```python
from build123d import *

# Parameters (mm, degrees)
SKETCH1_R           = 17.5
SKETCH1_R_2         = 10
BOSS_EXTRUDE1_DEPTH = 25
CUT_EXTRUDE1_START  = -10
SKETCH2_R           = 17.5
SKETCH2_R_2         = 15
CUT_EXTRUDE1_DEPTH  = 10
CHAMFER1_SIZE       = 1


with BuildPart() as part:
    # Sketch1 → Boss-Extrude1 (new body)
    with BuildSketch(Plane.XY):
        Circle(SKETCH1_R)
        Circle(SKETCH1_R_2, mode=Mode.SUBTRACT)
    extrude(amount=BOSS_EXTRUDE1_DEPTH)

    # Sketch2 → Cut-Extrude1 (cut)
    with BuildSketch(Plane.XY.offset(25).offset(CUT_EXTRUDE1_START)):
        Circle(SKETCH2_R)
        Circle(SKETCH2_R_2, mode=Mode.SUBTRACT)
    extrude(amount=CUT_EXTRUDE1_DEPTH, mode=Mode.SUBTRACT)

    # Chamfer1
    chamfer1_edges = [part.edges().sort_by_distance(p)[0] for p in [
        (-15, 0, 25),
    ]]
    chamfer(chamfer1_edges, length=CHAMFER1_SIZE)


solid = part.part
```
Design review of the part built by this model. Coordinates are the model's own, in mm. A direction names the side the tool comes from. Coordinates: 2 decimals unless noted, no trailing zeros. Order: outer loops, then holes, each group sorted by start corner. A loop starts at its lowest first (then second) coordinate and runs counter-clockwise, first axis right, second up.
1) Mouldability with a two-part tool opening along Y and no side actions: class faces 1 (the cylindrical face through (-2.17, -9.76, 12.32)), 2 (the flat face through (-10, 3, 25)), 3 (the cylindrical face through (-13.887, -10.648, 7.395)) as +Y half, -Y half, draft (parallel to the pull), parting line (faces both ways), or undercut.
2) Take a section at A-A, the plane y = 0. Give the boundary of the cut face in (x, z).
3) Wall thickness on line 1 along Y through (x, z) = (0, 11.75); line 2 along Z through (x, y) = (12, -10); line 3 along Y through (x, z) = (-2, 18): over which ranges is each line inside the solid? List them lowest first.
4) Clearance check with flat-ended pins moving along their axes: pin 1 (3 mm diameter, centred on x = -9.5, z = 5.5, fed in from -Y); pin 2 (1.5 mm diameter, centred on y = -13, z = 7, fed in from -X); pin 3 (4 mm diameter, centred on x = 12, z = 21, fed in from -Y). State where each tip first meets the part, or that it passes through.
5) For faces 4 (the flat face through (13, 8, 15)), 5 (the flat face through (8, -8, 0)), list the 3-axis set-ups (+Z, -Z, +X, -X, +Y, -Y) from which the entire face can be reached by the end or side of a thin tool; tool diameter is ignored.
6) Take a section at C-C, the plane z = 20. Give the boundary of the cut face in (x, y).
Returned:
1. face 1: undercut
1. face 2: draft
1. face 3: parting line
2. outline: (-17.5, 0) - (-10, 0) - (-10, 25) - (-14, 25) - (-15, 24) - (-15, 15) - (-17.5, 15) - close; (10, 0) - (17.5, 0) - (17.5, 15) - (15, 15) - (15, 24) - (14, 25) - (10, 25) - close
3. line 1: y = -17.5 to -10, 10 to 17.5
3. line 2: z = 0 to 15
3. line 3: y = -14.87 to -9.8, 9.8 to 14.87
4. pin 1: stops at y = -15.56
4. pin 2: stops at x = -12.5
4. pin 3: stops at y = -11.18
5. face 4: +Z
5. face 5: -Z, +X, -X, +Y, -Y
6. outline: circle Ø30 at (0, 0); hole circle Ø20 at (0, 0)
